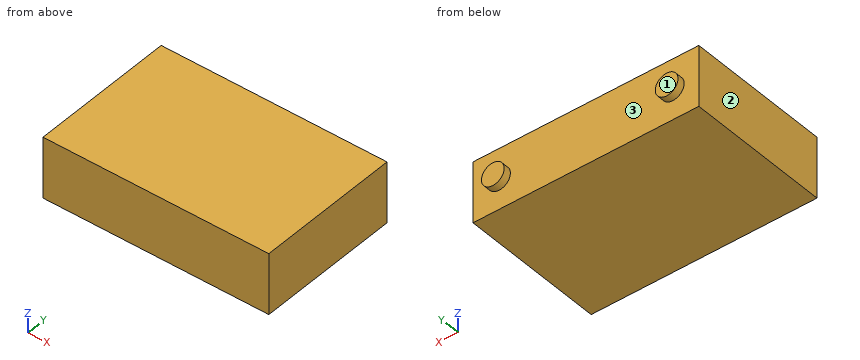
```python
from build123d import *

# Parameters (mm, degrees)
SKETCH_1_W      = 148.9
SKETCH_1_H      = 40.2
EXTRUDE_1_DEPTH = 95.6
SKETCH_2_R      = 7.5
EXTRUDE_2_DEPTH = 5


with BuildPart() as part:
    # 草图1 → 凸台-拉伸1 (new body)
    with BuildSketch(Plane(origin=(0, 0, 0), x_dir=(1, 0, 0), z_dir=(0, 1, 0))):
        Rectangle(SKETCH_1_W, SKETCH_1_H)
    extrude(amount=EXTRUDE_1_DEPTH)

    # 草图2 → 凸台-拉伸2 (add)
    with BuildSketch(Plane(origin=(0, 95.6, 0), x_dir=(1, 0, 0), z_dir=(0, 1, 0))):
        with Locations(Location((57.3, 0, 0), (0, 0, 270))):
            Circle(SKETCH_2_R)
        with Locations(Location((-57.3, 0, 0), (0, 0, 270))):
            Circle(SKETCH_2_R)
    extrude(amount=EXTRUDE_2_DEPTH)


solid = part.part
```
Verification items for the finished model (mm, model axes). Face numbers are marked on the shaded views. Round coordinates to 2 decimals unless told otherwise and drop trailing zeros. Order: outer loops, then holes, each group sorted by start corner. A loop starts at its lowest first (then second) coordinate and runs counter-clockwise, first axis right, second up.
1) Draft check along X on the marked faces 1, 2 and 3. Enter one of: +X half, -X half, draft (parallel to the pull), parting line (faces both ways), or undercut.
Geometry says:
face 1: draft
face 2: -X half
face 3: undercut
2) Cross-section at D-D, the plane z = -17. Record the cut outline in (x, y).
Geometry says:
outline: (-74.45, 0) - (74.45, 0) - (74.45, 95.6) - (-74.45, 95.6) - close
3) Cross-section at C-C, the plane x = 34. Record the cut outline in (y, z), plus the area to 3 significant figures.
Geometry says:
outline: (0, -20.1) - (95.6, -20.1) - (95.6, 20.1) - (0, 20.1) - close
area: 3,840 mm2
4) Depth check by flat-ended pin: pin 1 (20 mm diameter, centred on x = -10.5, z = 2.5, fed in from +Y). Enter the tip coordinate at first touch or a pass-through.
Geometry says:
pin 1: stops at y = 95.6
5) Cross-section at B-B, the plane z = 0. Record the cut outline in (x, y), plus the area to 3 significant figures.
Geometry says:
outline: (-74.45, 0) - (74.45, 0) - (74.45, 95.6) - (64.8, 95.6) - (64.8, 100.6) - (49.8, 100.6) - (49.8, 95.6) - (-49.8, 95.6) - (-49.8, 100.6) - (-64.8, 100.6) - (-64.8, 95.6) - (-74.45, 95.6) - close
area: 14,400 mm2
6) Cross-section at A-A, the plane x = -57.3. Record the cut outline in (y, z), plus the area to 3 significant figures.
Geometry says:
outline: (0, -20.1) - (95.6, -20.1) - (95.6, -7.5) - (100.6, -7.5) - (100.6, 7.5) - (95.6, 7.5) - (95.6, 20.1) - (0, 20.1) - close
area: 3,920 mm2
7) Material ranges on line 1 (Y direction, x = -38.5, z = -4), recorded low to high.
Geometry says:
line 1: y = 0 to 95.6
